Geometry: final body of the model. Coordinates: model frame, mm. Round coordinates to 2 decimals unless told otherwise and drop trailing zeros. Loops run counter-clockwise (first coordinate to the right, second up) from the corner with the lowest first, then second, coordinate; pieces in that order, holes last. Notation, with made-up numbers: M -11.75,1 L 9.25,1 A24 ccw 9.25,39 Z; hole C 7,33.5 d5. An arc over 180 degrees is marked long. Return JSON: item names as keys, results as strings.
from build123d import *

# Parameters (mm, degrees)
BOSS_EXTRUDE1_DEPTH = 14


with BuildPart() as part:
    # Sketch1 → Boss-Extrude1 (new body)
    with BuildSketch(Plane.XY):
        Polygon((-95.25, 755.65), (0, 755.65), (95.25, 755.65), (109.5375, 742.95), (117.475, 698.5), (366.7125, 9.525), (357.1875, 0), (0, 0), (-357.1875, 0), (-366.7125, 9.525), (-117.475, 698.5), (-109.5375, 742.95), align=None)
        Polygon((-280.465202582, 50.8), (280.465202582, 50.8), (293.165202582, 63.5), (65.476347176, 692.907409213), (48.4561012, 704.85), (-48.4561012, 704.85), (-65.476347176, 692.907409213), (-293.165202582, 63.5), align=None, mode=Mode.SUBTRACT)
    extrude(amount=BOSS_EXTRUDE1_DEPTH)


solid = part.part
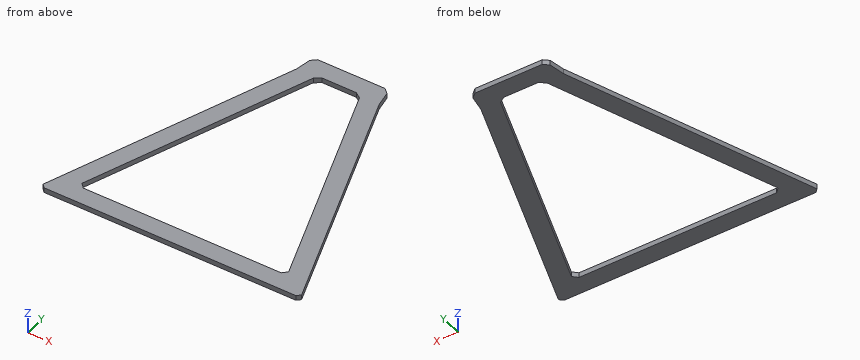
Q1. Pin query (flat end, axial travel): pin 1 (2 mm diameter, centred on y = 615, z = 6, fed in from +X). Return the tip coordinate at first contact, or that it passes through.
Determined:
{"pin 1": "stops at x = 148.04"}
Q2. Material intervals for L1, parallel to Y at x = 35, z = 8.25; L2, parallel to X at y = 293, z = 6.75; L3, parallel to X at y = 539.5, z = 9, sorted ascending.
Determined:
{"L1": "y = 0 to 50.8, 704.85 to 755.65", "L2": "x = -264.17 to -210.14, 210.14 to 264.17", "L3": "x = -174.99 to -120.97, 120.97 to 174.99"}
Q3. Section query B-B (x = 81). Output: boundary loops of the cut face in (y, z), plus the area to 3 significant figures.
Determined:
{"outline": "M 0,0 L 50.8,0 L 50.8,14 L 0,14 Z; M 649.99,0 L 755.65,0 L 755.65,14 L 649.99,14 Z", "area": "2,190 mm^2"}
Q4. Section query C-C (y = 481.5). Output: boundary loops of the cut face in (x, z) (3 decimals), plus the area to 3 significant figures.
Determined:
{"outline": "M -195.975,0 L -141.953,0 L -141.953,14 L -195.975,14 Z; M 141.953,0 L 195.975,0 L 195.975,14 L 141.953,14 Z", "area": "1,510 mm^2"}
Q5. Section query D-D (x = 318). Output: boundary loops of the cut face in (y, z).
Determined:
{"outline": "M 0,0 L 144.18,0 L 144.18,14 L 0,14 Z"}
